from build123d import *

# Parameters (mm, degrees)
BRACKET_PROFILE_SKETCH_W = 44
BRACKET_PROFILE_SKETCH_H = 55.25
BRACKET_BODY_DEPTH       = 45
BEARING_SEAT_R25_DEPTH   = 45
BASE_SLOT_SKETCH_W       = 16.5
BASE_SLOT_SKETCH_H       = 50
BASE_MOUNTING_SLOT_DEPTH = 11
TOP_RECESSES_DEPTH       = 15


with BuildPart() as part:
    # Bracket Profile Sketch → Bracket Body (new, symmetric)
    with BuildSketch(Plane.XY):
        with Locations((22, 27.625)):
            Rectangle(BRACKET_PROFILE_SKETCH_W, BRACKET_PROFILE_SKETCH_H)
        Polygon((44, 22), (44, 0), (70.5, 0), (70.5, 11), (64, 22), align=None)
    extrude(amount=BRACKET_BODY_DEPTH, both=True)

    # Bearing Seat Sketch → Bearing Seat R25 (cut)
    with BuildSketch(Plane(origin=(44, 0, 0), x_dir=(0, 0, -1), z_dir=(1, 0, 0))):
        with BuildLine():
            Line((-25, 55.25), (25, 55.25))
            ThreePointArc((25, 55.25), (0, 30.25), (-25, 55.25))
        make_face()
    extrude(amount=-BEARING_SEAT_R25_DEPTH, mode=Mode.SUBTRACT)

    # Base Slot Sketch → Base Mounting Slot (cut)
    with BuildSketch(Plane(origin=(0, 22, 0), x_dir=(1, 0, 0), z_dir=(0, 1, 0))):
        with Locations((62.25, 0)):
            Rectangle(BASE_SLOT_SKETCH_W, BASE_SLOT_SKETCH_H)
    extrude(amount=-BASE_MOUNTING_SLOT_DEPTH, mode=Mode.SUBTRACT)

    # Top Recess Sketch → Top Recesses (cut)
    with BuildSketch(Plane(origin=(0, 55.25, 0), x_dir=(1, 0, 0), z_dir=(0, 1, 0))):
        Polygon((9.5, -33.5), (22, -33.5), (34.5, -33.5), (34.5, -18.5), (9.5, -18.5), align=None)
        Polygon((22, 33.5), (34.5, 33.5), (34.5, 18.5), (9.5, 18.5), (9.5, 33.5), align=None)
    extrude(amount=-TOP_RECESSES_DEPTH, mode=Mode.SUBTRACT)


solid = part.part
Read the model definition and answer for the solid it produces. Units are mm, in the model's axes. A direction names the side the tool comes from. Give positions to 0.01 mm unless a question says otherwise; leave off trailing zeros. Write each loop counter-clockwise with the first axis right and the second up, starting at its lowest first coordinate (ties: lowest second). Pieces come first, ordered by that corner, then holes. Notation, with made-up numbers: (72, 65) - (121, 65) arc R11 ccw to (121, 69) - close; hole circle Ø8 at (74, -4). An arc over 180 degrees is marked (long way). Return JSON: item names as keys, results as strings.
Q1. For faces 1 (the face through (22, 48, 33.5)), 2 (the face through (62, 11, 0)), 3 (the face through (27, 28, 45)), determine the directions among +Z, -Z, +X, -X, +Y, -Y from which every point of the face is accessible in a straight line to the end or side of a thin tool.
Reply:
{"face 1": "+Y", "face 2": "+X, +Y", "face 3": "+Z, +X, -X, +Y, -Y"}
Q2. Given P1, Ø22, axis at x = 53.5, z = -7, coming from the +Y side; P2, Ø11, axis at y = 51, z = 25, coming from the +X side; P3, Ø11, axis at x = 16.5, z = -25, coming from the +Y side, each flat-ended and moving along its own axis, determine where each tip first touches the part or whether it passes through.
Reply:
{"P1": "y = 33.63", "P2": "x = 44", "P3": "y = 40.25"}
Q3. A cutting plane is placed at D-D, the plane y = 26. Determine the outline of the cut face in (x, z), and give its area (3 significant figures).
Reply:
{"outline": "(0, -45) - (44, -45) - (44, 45) - (0, 45) - close", "area": "3,960 mm²"}
Q4. A cutting plane is placed at B-B, the plane z = 0. Determine the outline of the cut face in (x, y).
Reply:
{"outline": "(0, 0) - (70.5, 0) - (70.5, 11) - (54, 11) - (54, 22) - (44, 22) - (44, 30.25) - (0, 30.25) - close"}
Q5. A cutting plane is placed at A-A, the plane y = 36.5. Determine the outline of the cut face in (x, z).
Reply:
{"outline": "(0, -45) - (44, -45) - (44, -16.54) - (0, -16.54) - close; (0, 16.54) - (44, 16.54) - (44, 45) - (0, 45) - close"}
Q6. For a pull along X with two mould halves and no side action, classify faces 4 (the face through (0, 21, 1)), 5 (the face through (52, 22, 1)), 6 (the face through (22, 48, -33.5)), 7 (the face through (22, 40.25, 27)) as released by +X, released by -X, zero draft, split by the parting line, or undercut.
Reply:
{"face 4": "released by -X", "face 5": "zero draft", "face 6": "undercut", "face 7": "undercut"}
Q7. A cutting plane is placed at C-C, the plane x = 56. Determine the outline of the cut face in (y, z).
Reply:
{"outline": "(0, -45) - (22, -45) - (22, -25) - (11, -25) - (11, 25) - (22, 25) - (22, 45) - (0, 45) - close"}
Q8. Consider line 1 along Z through (x, y) = (13, 42.5); line 2 along X through (y, z) = (32, 16); line 3 along X through (y, z) = (21, 8.5). Determine where each line is inside the solid, lowest interval first. Write a range as [from, to].
Reply:
{"line 1": "[-45, -33.5], [33.5, 45]", "line 2": "[0, 44]", "line 3": "[0, 54]"}
